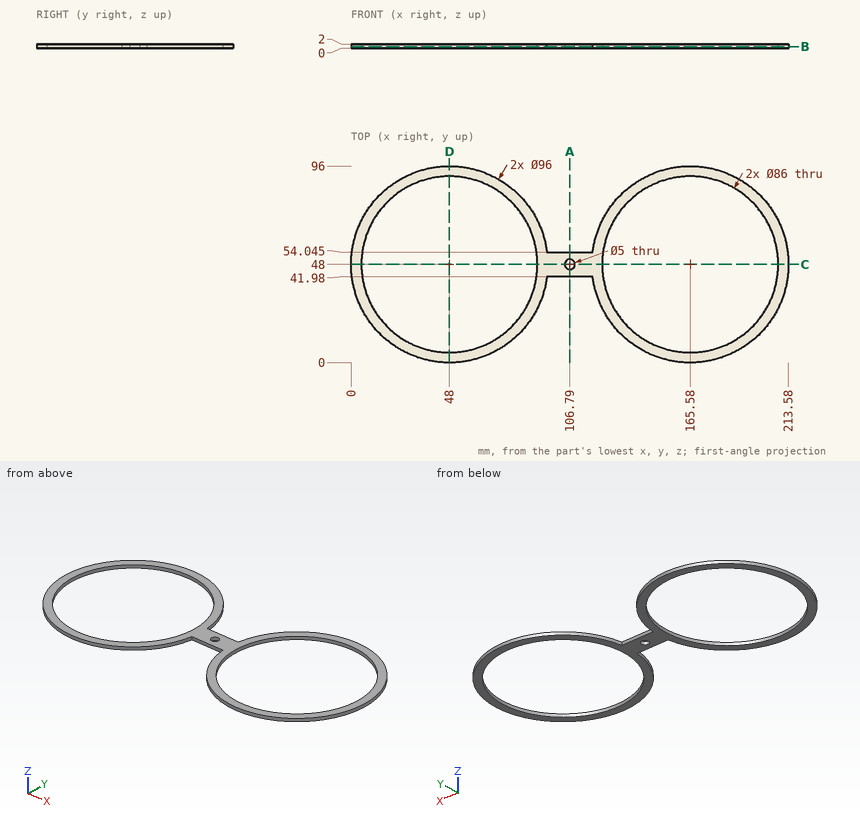
Here's the drawing with two shaded views (mm, measured from the low corner). I have some questions. Round coordinates to 2 decimals unless told otherwise and drop trailing zeros. Loops run counter-clockwise (first coordinate to the right, second up) from the corner with the lowest first, then second, coordinate; pieces in that order, holes last. Notation, with made-up numbers: M -4,56.25 L 29,56.25 A24 ccw 29,83.25 Z; hole C 15,67.5 d7. An arc over 180 degrees is marked long. Answer as CSV lines item,"result".
1) Imagine slicing it at D-D on x = 48. List the corners of the cut face in (y, z) for me.
From the geometry:
outline,"M 0,0 L 5,0 L 5,2 L 0,2 Z; M 91,0 L 96,0 L 96,2 L 91,2 Z"
2) Imagine slicing it at A-A on x = 106.79. List the corners of the cut face in (y, z) for me (1 decimal), and give its area (3 significant figures).
From the geometry:
outline,"M 42,0 L 45.5,0 L 45.5,2 L 42,2 Z; M 50.5,0 L 54,0 L 54,2 L 50.5,2 Z"
area,"14.1 mm^2"
3) For pin 1 Ø1 at (x, z) = (115, 0.5) entering from +Y (1 decimal); pin 2 Ø0.6 at (x, z) = (107.5, 1) entering from -Y, each with a flat end and sliding along its axis, tell me the tip position at first contact or that it passes through.
From the geometry:
pin 1,"y = 54"
pin 2,"y = 41.98"
4) Imagine slicing it at C-C on y = 48. List the corners of the cut face in (x, z) for me.
From the geometry:
outline,"M 0,0 L 5,0 L 5,2 L 0,2 Z; M 91,0 L 104.29,0 L 104.29,2 L 91,2 Z; M 109.29,0 L 122.58,0 L 122.58,2 L 109.29,2 Z; M 208.58,0 L 213.58,0 L 213.58,2 L 208.58,2 Z"
5) Imagine slicing it at B-B on z = 0.7. List the corners of the cut face in (x, y) for me (1 decimal).
From the geometry:
outline,"M 95.6,42 L 118,42 A48 ccw long 118,54 L 95.6,54 A48 ccw long Z; hole C 48,48 d86; hole C 106.8,48 d5; hole C 165.6,48 d86"
6) If I drill on probe 1 along X at (y, z) = (48, 0.9); probe 2 along Y at (x, z) = (106.79, 0.75) (1 decimal); probe 3 along Y at (x, z) = (165.58, 0.95), over which ranges is the centre line in solid material (lowest first)?
From the geometry:
probe 1,"0 to 5, 91 to 104.29, 109.29 to 122.58, 208.58 to 213.58"
probe 2,"42 to 45.5, 50.5 to 54"
probe 3,"0 to 5, 91 to 96"
